Here's the drawing with two shaded views (mm, measured from the low corner). I have some questions. A direction names the side the tool comes from. Give positions to 0.01 mm unless a question says otherwise; leave off trailing zeros. Loops run counter-clockwise (first coordinate to the right, second up) from the corner with the lowest first, then second, coordinate; pieces in that order, holes last. Notation, with made-up numbers: M 56.25,1.5 L 107.25,1.5 A26 cw 107.25,39.5 Z; hole C 27.5,72.5 d7. An arc over 180 degrees is marked long. Put each result on its own line as item: value. Start each with the question number.
1) For P1, Ø4, axis at x = 14.5, z = 29, coming from the -Y side; P2, Ø3, axis at y = 74.5, z = 21, coming from the +X side; P3, Ø6, axis at y = 68, z = 19, coming from the +X side, each with a flat end and sliding along its axis, tell me the tip position at first contact or that it passes through.
2) Imagine slicing it at A-A (x = 44.5). Write out the boundary of the cut face in (y, z).
3) Imagine slicing it at D-D (z = 7). Write out the boundary of the cut face in (x, y), then the cut area to 3 significant figures.
4) For the marked faces 1 and 2, which set-ups out of +Z, -Z, +X, -X, +Y, -Y let a thin tool reach every point of the face, with its end or its side?
5) Imagine slicing it at C-C (z = 42). Write out the boundary of the cut face in (x, y).
6) Please list where these lines run through material, in increasing order: line 1 along Y through (x, z) = (44.5, 29); line 2 along X through (y, z) = (44, 68); line 3 along Y through (x, z) = (60.5, 22.5). Write a range as from..to.
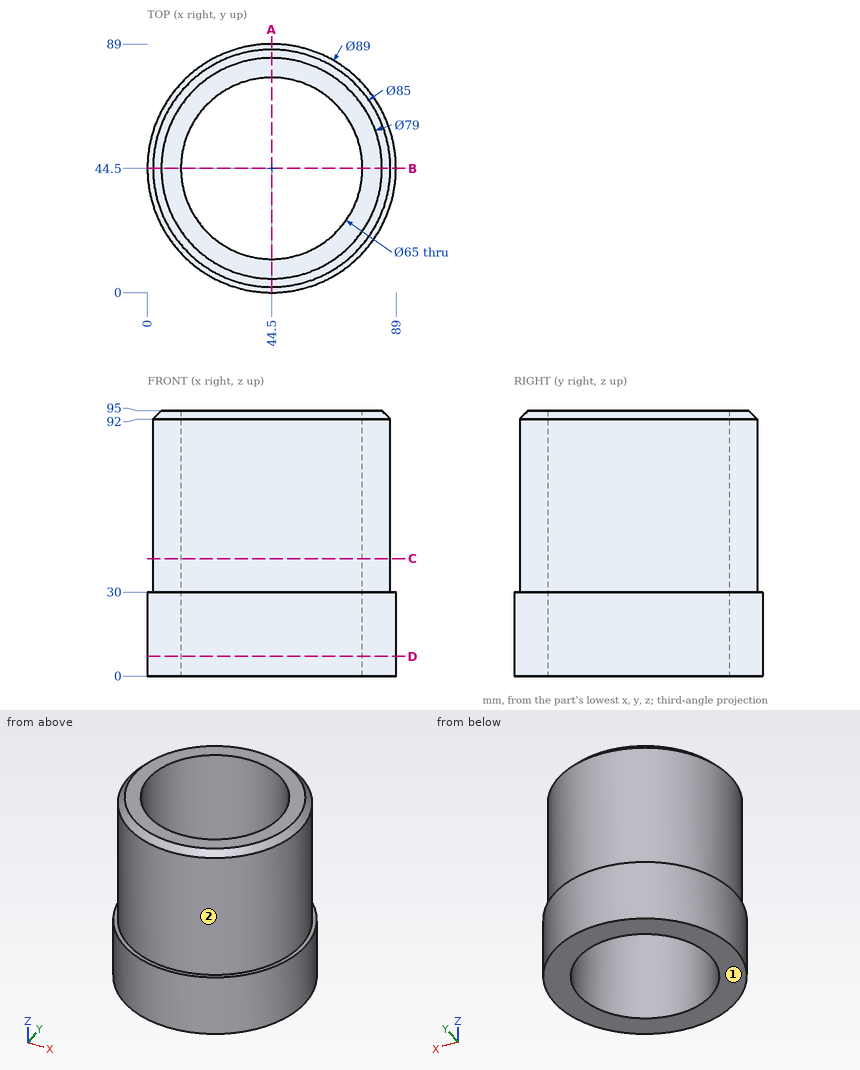
Recorded:
1. P1: y = 9.91
1. P2: x = 78.68
1. P3: x = 84
2. outline: M 0,0 L 12,0 L 12,95 L 5,95 L 2,92 L 2,30 L 0,30 Z; M 77,0 L 89,0 L 89,30 L 87,30 L 87,92 L 84,95 L 77,95 Z
3. outline: C 44.5,44.5 d89; hole C 44.5,44.5 d65
3. area: 2,900 mm²
4. face 1: -Z, +X, -X, +Y, -Y
4. face 2: +Z
5. outline: C 44.5,44.5 d85; hole C 44.5,44.5 d65
6. line 1: 0..12, 77..89
6. line 2: 2..12, 77..87
6. line 3: 2.98..16.21, 72.79..86.02
